```python
from build123d import *

# Parameters (mm, degrees)
SKETCH1_W          = 50
SKETCH1_H          = 124
EXTRUDE1_DEPTH     = 3
SKETCH2_R          = 6.5
CUT_EXTRUDE1_DEPTH = 22


with BuildPart() as part:
    # Sketch1 → Extrude1 (new, symmetric)
    with BuildSketch(Plane.XY):
        Rectangle(SKETCH1_W, SKETCH1_H)
    extrude(amount=EXTRUDE1_DEPTH, both=True)

    # Sketch2 → Cut-Extrude1 (cut)
    with BuildSketch(Plane.XY.offset(3)):
        with Locations((0, 30)):
            Circle(SKETCH2_R)
        with Locations((0, -30)):
            Circle(SKETCH2_R)
    extrude(amount=-CUT_EXTRUDE1_DEPTH, mode=Mode.SUBTRACT)


solid = part.part
```
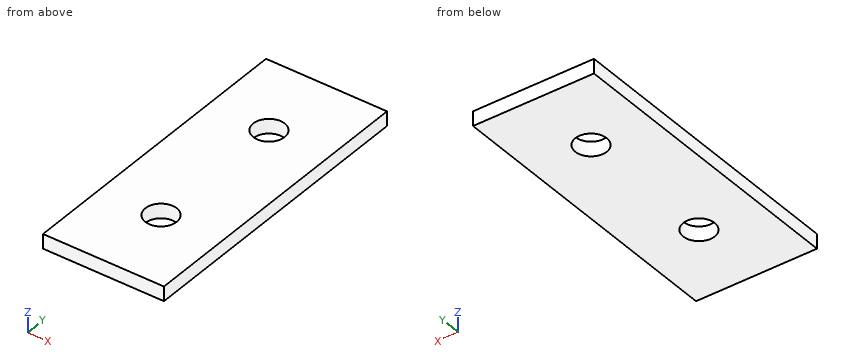
Verification items for the finished model (mm, model axes). Round coordinates to 2 decimals unless told otherwise and drop trailing zeros. Write each loop counter-clockwise with the first axis right and the second up, starting at its lowest first coordinate (ties: lowest second). Pieces come first, ordered by that corner, then holes. Notation, with made-up numbers: (79, -23) -> (85, -23) arc R28 cw to (85, 5) -> close; hole circle Ø4 at (-14.75, 48.25). An arc over 180 degrees is marked (long way). Write each question's results on one line, items separated by ' | '. Start each with the question number.
1. Cross-section at C-C (z = -1). Enter the section's corners in (x, y), then the cut area to 3 significant figures.
2. Cross-section at B-B (x = 0). Enter the section's corners in (y, z), then the cut area to 3 significant figures.
3. Cross-section at A-A (y = 30). Enter the section's corners in (x, z).
4. Material ranges on probe 1 along Y at (x, z) = (0, 1.6); probe 2 along X at (y, z) = (30.5, -0.05); probe 3 along Y at (x, z) = (-4, -0.6), recorded low to high. Write a range as from..to.
5. Depth check by flat-ended pin: P1, Ø10.5, axis at x = 0, y = 30, coming from the -Z side. Enter the tip coordinate at first touch or a pass-through.
Solutions:
1) outline: (-25, -62) -> (25, -62) -> (25, 62) -> (-25, 62) -> close; hole circle Ø13 at (0, -30); hole circle Ø13 at (0, 30) | area: 5,930 mm2
2) outline: (-62, -3) -> (-36.5, -3) -> (-36.5, 3) -> (-62, 3) -> close; (-23.5, -3) -> (23.5, -3) -> (23.5, 3) -> (-23.5, 3) -> close; (36.5, -3) -> (62, -3) -> (62, 3) -> (36.5, 3) -> close | area: 588 mm2
3) outline: (-25, -3) -> (-6.5, -3) -> (-6.5, 3) -> (-25, 3) -> close; (6.5, -3) -> (25, -3) -> (25, 3) -> (6.5, 3) -> close
4) probe 1: y = -62..-36.5, -23.5..23.5, 36.5..62 | probe 2: x = -25..-6.48, 6.48..25 | probe 3: y = -62..-35.12, -24.88..24.88, 35.12..62
5) P1: passes through
